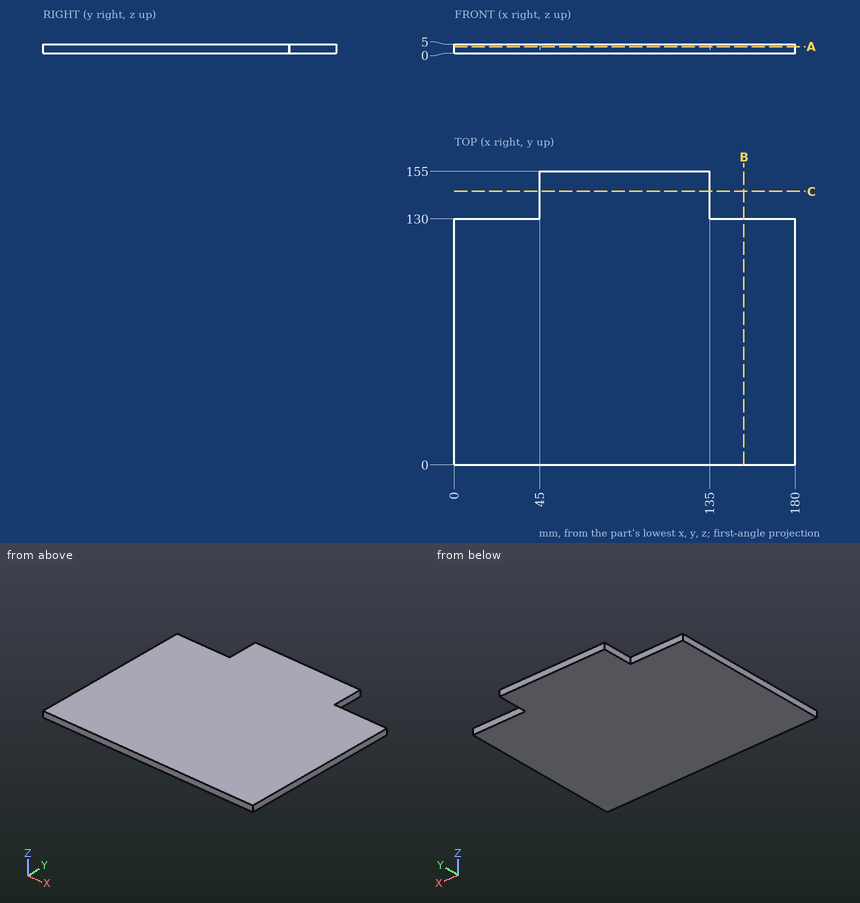
Verification items for this drawing (mm, ordinates from the low corner). Coordinates: 2 decimals unless noted, no trailing zeros. Order: outer loops, then holes, each group sorted by start corner. A loop starts at its lowest first (then second) coordinate and runs counter-clockwise, first axis right, second up. Notation, with made-up numbers: M -26.5,81.25 L 20.5,81.25 A15 cw 20.5,106.25 Z; hole C 45.25,-38 d2. An arc over 180 degrees is marked long. One line per item, written item: value. Start each with the question number.
Item 1: Depth check by flat-ended pin: P1, Ø2.5, axis at x = 18.5, z = 2.5, coming from the +Y side; P2, Ø1.5, axis at y = 136.5, z = 3, coming from the -X side. Enter the tip coordinate at first touch or a pass-through.
Item 2: Sectioned sample at B-B on x = 153. Record the cut outline in (y, z), then the cut area to 3 significant figures.
Item 3: Thickness scan on probe 1 along Y at (x, z) = (38, 0.6); probe 2 along X at (y, z) = (140, 3.5). Record the ranges inside material, lowest first.
Item 4: Sectioned sample at A-A on z = 3.55. Record the cut outline in (x, y), then the cut area to 4 significant figures.
Item 5: Sectioned sample at C-C on y = 144.5. Record the cut outline in (x, z), then the cut area to 3 significant figures.
Calculated:
1. P1: y = 130
1. P2: x = 45
2. outline: M 0,0 L 130,0 L 130,5 L 0,5 Z
2. area: 650 mm^2
3. probe 1: 0 to 130
3. probe 2: 45 to 135
4. outline: M 0,0 L 180,0 L 180,130 L 135,130 L 135,155 L 45,155 L 45,130 L 0,130 Z
4. area: 25,650 mm^2
5. outline: M 45,0 L 135,0 L 135,5 L 45,5 Z
5. area: 450 mm^2
